Verification items for this drawing (mm, ordinates from the low corner). Coordinates: 2 decimals unless noted, no trailing zeros. Order: outer loops, then holes, each group sorted by start corner. A loop starts at its lowest first (then second) coordinate and runs counter-clockwise, first axis right, second up. Notation, with made-up numbers: (7.5, 54) -> (32.5, 54) arc R8 cw to (32.5, 67) -> close; hole circle Ø3 at (65.5, 87). An arc over 180 degrees is marked (long way). Write item = value, one per line. Start each with the question number.
1. Release check for a two-part mould opening along Z. For the marked faces 1, 2 and 3 record: +Z half, -Z half, draft (parallel to the pull), parting line (faces both ways), or undercut.
2. Cross-section at A-A on z = 20. Record the cut outline in (x, y), plus the area to 3 significant figures.
3. Cross-section at C-C on y = 1.8. Record the cut outline in (x, z), plus the area to 3 significant figures.
4. Thickness scan on line 1 along X through (y, z) = (1.4, 20); line 2 along X through (y, z) = (1.6, 35); line 3 along X through (y, z) = (5.45, 8.5). Record the ranges inside material, lowest first. Write a range as from..to.
5. Cross-section at B-B on x = 75. Record the cut outline in (y, z).
6. Go/stop test with a flat-tipped pin: P1, Ø8.5, axis at x = 75, z = 20, coming from the +Y side. Record where the tip stops, or that it passes through.
7. Cross-section at D-D on z = 35.5. Record the cut outline in (x, y), plus the area to 3 significant figures.
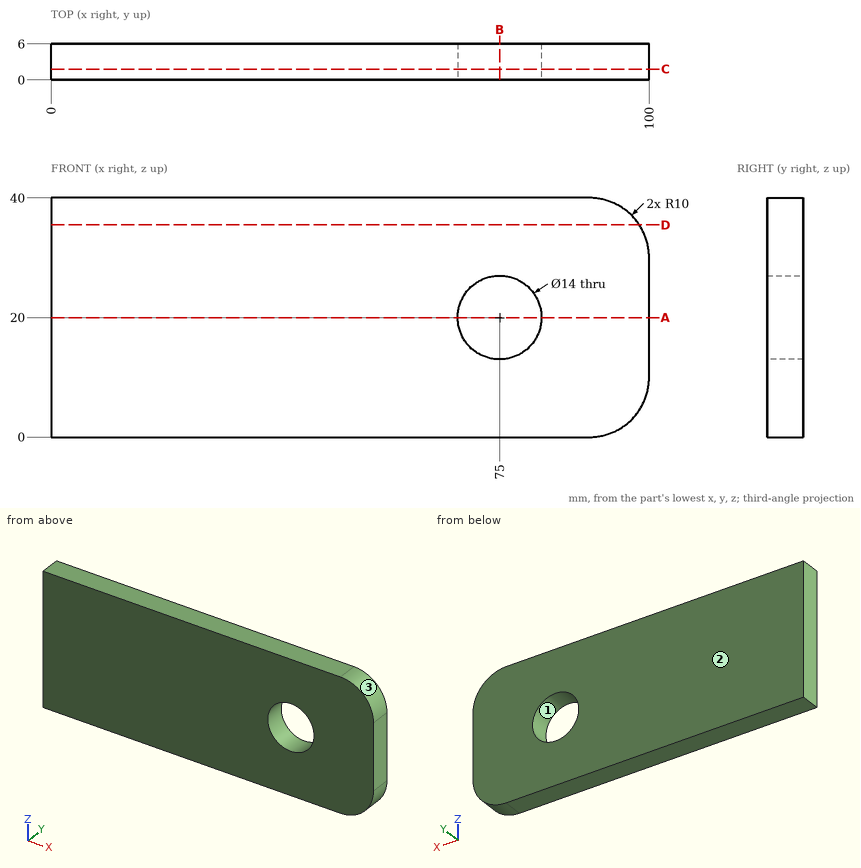
Worked out:
q1.face_1 = undercut
q1.face_2 = draft
q1.face_3 = +Z half
q2.outline = (0, 0) -> (68, 0) -> (68, 6) -> (0, 6) -> close; (82, 0) -> (100, 0) -> (100, 6) -> (82, 6) -> close
q2.area = 516 mm²
q3.outline = (0, 0) -> (90, 0) arc R10 ccw to (100, 10) -> (100, 30) arc R10 ccw to (90, 40) -> (0, 40) -> close; hole circle Ø14 at (75, 20)
q3.area = 3,800 mm²
q4.line_1 = 0..68, 82..100
q4.line_2 = 0..98.66
q4.line_3 = 0..99.89
q5.outline = (0, 0) -> (6, 0) -> (6, 13) -> (0, 13) -> close; (0, 27) -> (6, 27) -> (6, 40) -> (0, 40) -> close
q6.P1 = through
q7.outline = (0, 0) -> (98.35, 0) -> (98.35, 6) -> (0, 6) -> close
q7.area = 590 mm²
